Verification items for the finished model (mm, model axes). Coordinates: 2 decimals unless noted, no trailing zeros. Write each loop counter-clockwise with the first axis right and the second up, starting at its lowest first coordinate (ties: lowest second). Pieces come first, ordered by that corner, then holes. Notation, with made-up numbers: (-30.5, -16.5) -> (3.5, -16.5) arc R22 cw to (3.5, -5.5) -> close; hole circle Ø2 at (-27, -20). An arc over 180 degrees is marked (long way). Use CSV: the item, a comma, the result in double quotes.
```python
from build123d import *

# Parameters (mm, degrees)
SKETCH_1_W                = 80
SKETCH_1_H                = 350
EXTRUDE_1_DEPTH           = 10
HOLE_WIZARD_M5_1_D        = 4.2
HOLE_WIZARD_1_D           = 6.6
HOLE_WIZARD_1_CBORE_D     = 11
HOLE_WIZARD_1_CBORE_DEPTH = 6.8
CUT_EXTRUDE_1_REACH       = 181.792
SKETCH_6_R                = 20
PATTERN_LINEAR_1_COUNT    = 3
PATTERN_LINEAR_1_PITCH    = 100


with BuildPart() as part:
    # 草图1 → 凸台-拉伸1 (new body)
    with BuildSketch(Plane.XY):
        Rectangle(SKETCH_1_W, SKETCH_1_H)
    extrude(amount=EXTRUDE_1_DEPTH)

    # M5 螺纹孔1 (through all)
    with Locations(Plane(origin=(0, 0, 0), x_dir=(-1, 0, 0), z_dir=(0, 0, -1))):
        with Locations((-33.000000411, 150), (34.999999589, 150), (-33.000000411, 50), (34.999999589, 50), (-33.000000411, -50), (34.999999589, -50), (-33.000000411, -150), (34.999999589, -150)):
            Hole(HOLE_WIZARD_M5_1_D / 2)

    # 打孔尺寸(%根据)内六角圆柱头螺钉的类型1 (through all)
    with Locations(Plane(origin=(0, 0, 0), x_dir=(-1, 0, 0), z_dir=(0, 0, -1))):
        with Locations((-20, 40), (20, 40), (20, -40), (-20, -40)):
            CounterBoreHole(HOLE_WIZARD_1_D / 2, HOLE_WIZARD_1_CBORE_D / 2, HOLE_WIZARD_1_CBORE_DEPTH)

    # 草图6 → 切除-拉伸1 (cut, up to next)
    with BuildSketch(Plane(origin=(0, 0, 0), x_dir=(-1, 0, 0), z_dir=(0, 0, -1)), mode=Mode.PRIVATE) as cut_extrude_1_sk1:
        with Locations((0, -105)):
            Circle(SKETCH_6_R)
    cut_extrude_1_tool1 = extrude(cut_extrude_1_sk1.sketch, amount=-CUT_EXTRUDE_1_REACH, mode=Mode.PRIVATE) & part.part
    cut_extrude_1 = cut_extrude_1_tool1.solids().sort_by_distance((0, -105, 0))[0]
    add(cut_extrude_1, mode=Mode.SUBTRACT)

    # 阵列(线性)1: 切除-拉伸1 ×3
    with Locations(*[(0, i * PATTERN_LINEAR_1_PITCH, 0) for i in range(1, PATTERN_LINEAR_1_COUNT)]):
        add(cut_extrude_1, mode=Mode.SUBTRACT)


solid = part.part
```
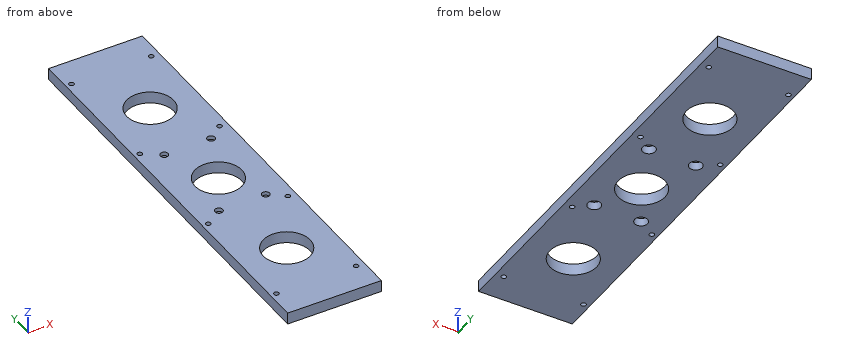
1) Cross-section at A-A (x = 0). Record the boundary of the cut face in (y, z).
Return value:
outline,"(-175, 0) -> (-125, 0) -> (-125, 10) -> (-175, 10) -> close; (-85, 0) -> (-25, 0) -> (-25, 10) -> (-85, 10) -> close; (15, 0) -> (75, 0) -> (75, 10) -> (15, 10) -> close; (115, 0) -> (175, 0) -> (175, 10) -> (115, 10) -> close"
2) Cross-section at C-C (y = -40). Record the boundary of the cut face in (x, z), plus the area to 3 significant figures.
Return value:
outline,"(-40, 0) -> (-25.5, 0) -> (-25.5, 6.8) -> (-23.3, 6.8) -> (-23.3, 10) -> (-40, 10) -> close; (-16.7, 6.8) -> (-14.5, 6.8) -> (-14.5, 0) -> (14.5, 0) -> (14.5, 6.8) -> (16.7, 6.8) -> (16.7, 10) -> (-16.7, 10) -> close; (23.3, 6.8) -> (25.5, 6.8) -> (25.5, 0) -> (40, 0) -> (40, 10) -> (23.3, 10) -> close"
area,"608 mm2"
3) Scan lines: L1, parallel to Y at x = 1.5, z = 9.25; L2, parallel to X at y = -150, z = 6.5; L3, parallel to Y at x = 0, z = 6.5. Record each from-to range of solid material in increasing order.
Return value:
L1,"-175 to -124.94, -85.06 to -24.94, 14.94 to 75.06, 114.94 to 175"
L2,"-40 to -37.1, -32.9 to 30.9, 35.1 to 40"
L3,"-175 to -125, -85 to -25, 15 to 75, 115 to 175"
4) Cross-section at D-D (y = 110). Record the boundary of the cut face in (x, z).
Return value:
outline,"(-40, 0) -> (-13.23, 0) -> (-13.23, 10) -> (-40, 10) -> close; (13.23, 0) -> (40, 0) -> (40, 10) -> (13.23, 10) -> close"
5) Gauge pin test, flat ends, axial feed: pin 1 (2.5 mm diameter, centred on x = -35, y = -150, fed in from -Z); pin 2 (5.5 mm diameter, centred on x = -18.5, y = 38.5, fed in from -Z). Record the tip position at first contact, or that the pin passes through.
Return value:
pin 1,"through"
pin 2,"z = 6.8"
6) Cross-section at B-B (z = 4.5). Give the number of separate pieces and of enclosed holes in the cut face, plus the area to 3 significant figures.
Return value:
separate pieces,"1"
enclosed holes,"15"
area,"23,700 mm2"
